from build123d import *

# Parameters (mm, degrees)
SKETCH1_W           = 270
SKETCH1_H           = 270
SKETCH1_W_2         = 250
SKETCH1_H_2         = 250
EXTRUDE_THIN1_DEPTH = 1000


with BuildPart() as part:
    # Sketch1 → Extrude-Thin1 (new body)
    with BuildSketch(Plane.XY):
        Rectangle(SKETCH1_W, SKETCH1_H)
        Rectangle(SKETCH1_W_2, SKETCH1_H_2, mode=Mode.SUBTRACT)
    extrude(amount=EXTRUDE_THIN1_DEPTH)


solid = part.part
CAD build for the part. Positions are in the model's coordinates, mm. A direction names the side the tool comes from. Coordinates: 2 decimals unless noted, no trailing zeros. Order: outer loops, then holes, each group sorted by start corner. A loop starts at its lowest first (then second) coordinate and runs counter-clockwise, first axis right, second up.
Item 1: Band-saw the part on A-A on z = 248.5. List the corners of the cut face in (x, y).
Check sheet entries:
outline: (-135, -135) - (135, -135) - (135, 135) - (-135, 135) - close; hole (-125, -125) - (125, -125) - (125, 125) - (-125, 125) - close
Item 2: Two-plate mould, pull along X, no slides. Class faces 1 (the face through (-135, -2, 493)), 2 (the face through (-2, 135, 493)), 3 (the face through (-125, -2, 493)): +X half, -X half, draft (parallel to the pull), parting line (faces both ways), or undercut.
Check sheet entries:
face 1: -X half
face 2: draft
face 3: undercut
Item 3: Band-saw the part on B-B on y = -14.5. List the corners of the cut face in (x, z).
Check sheet entries:
outline: (-135, 0) - (-125, 0) - (-125, 1000) - (-135, 1000) - close; (125, 0) - (135, 0) - (135, 1000) - (125, 1000) - close
Item 4: Drill centre line: L1, parallel to X at y = -14.5, z = 99. Where is it in solid material? Low to high.
Check sheet entries:
L1: x = -135 to -125, 125 to 135
Item 5: 3-axis set-ups, long thin cutter, end or side, ignore diameter. For faces 4 (the face through (-11, -129, 0)), 5 (the face through (-2, -125, 493)): which of +Z, -Z, +X, -X, +Y, -Y reach the whole face in a straight line?
Check sheet entries:
face 4: -Z, +X, -X, +Y, -Y
face 5: +Z, -Z
